from build123d import *

# Parameters (mm, degrees)
CHAMFER1_SIZE = 2


with BuildPart() as part:
    # Sketch1 → Revolve1 (revolve)
    with BuildSketch(Plane.XY, mode=Mode.PRIVATE) as revolve1_sk:
        Polygon((-30, 0), (-30, 33), (-38, 33), (-38, 8), (-55, 8), (-55, 0), align=None)
    revolve(revolve1_sk.sketch.rotate(Axis((0, 0, 0), (0, 1, 0)), 270), axis=Axis((0, 0, 0), (0, 1, 0)))

    # Chamfer1
    chamfer1_edges = [part.edges().sort_by_distance(p)[0] for p in [
        (0, 0, 55),
        (0, 33, 30),
        (0, 0, 30),
    ]]
    chamfer(chamfer1_edges, length=CHAMFER1_SIZE)


solid = part.part
Part model, mm, in its own coordinate system. A direction names the side the tool comes from. Coordinates: 2 decimals unless noted, no trailing zeros. Order: outer loops, then holes, each group sorted by start corner. A loop starts at its lowest first (then second) coordinate and runs counter-clockwise, first axis right, second up. Notation, with made-up numbers: M -27,-23 L -8,-23 A11 ccw -8,-9 Z; hole C 29,13.5 d3. An arc over 180 degrees is marked long. One line per question, with ' | ' between items.
Q1. Pin check, flat tips, straight feed: P1, Ø5, axis at x = 32.5, y = 29, coming from the -Z side; P2, Ø4, axis at x = 19, y = 9, coming from the +Z side; P3, Ø6, axis at x = 36, y = 17, coming from the -Z side. Stop position of each tip, or through.
A:
P1: stops at z = -23.32 | P2: stops at z = 52.22 | P3: stops at z = -18.84
Q2. Drill centre lines: line 1 (X direction, y = 9.5, z = 0); line 2 (Y direction, x = 32.5, z = -21); line 3 (X direction, y = 8.5, z = 25.5). Where is each one in solid material? Low to high.
A:
line 1: x = -38 to -30, 30 to 38 | line 2: y = 0 to 8 | line 3: x = -28.17 to -15.8, 15.8 to 28.17
Q3. Slice it at A-A (x = 0). Give the cut face in (y, z).
A:
outline: M 0,-53 L 2,-55 L 8,-55 L 8,-38 L 33,-38 L 33,-32 L 31,-30 L 2,-30 L 0,-32 Z; M 0,32 L 2,30 L 31,30 L 33,32 L 33,38 L 8,38 L 8,55 L 2,55 L 0,53 Z
Q4. Slice it at B-B (z = 0). Give the cut face in (x, y).
A:
outline: M -55,2 L -53,0 L -32,0 L -30,2 L -30,31 L -32,33 L -38,33 L -38,8 L -55,8 Z; M 30,2 L 32,0 L 53,0 L 55,2 L 55,8 L 38,8 L 38,33 L 32,33 L 30,31 Z
Q5. Two-plate mould, pull along X, no slides. Class faces 3 (the face through (-13, 8, 36)), 4 (the face through (48.794, 4.958, -25.379)), 5 (the face through (-1.32, 16.7, 29.97)): +X half, -X half, draft (parallel to the pull), parting line (faces both ways), or undercut.
A:
face 3: draft | face 4: parting line | face 5: undercut
Q6. 3-axis set-ups, long thin cutter, end or side, ignore diameter. For faces 1 (the face through (23.122, 20.325, 30.156)), 2 (the face through (11.54, 1.87, -27.83)): which of +Z, -Z, +X, -X, +Y, -Y reach the whole face in a straight line?
A:
face 1: +Y | face 2: -Y
Q7. Slice it at C-C (y = 18). Give the cut face in (x, z).
A:
outline: C 0,0 d76; hole C 0,0 d60
